Drawing for the job (mm, zero at the part's lowest x, y, z). A direction names the side the tool comes from. Coordinates: 2 decimals unless noted, no trailing zeros. Order: outer loops, then holes, each group sorted by start corner. A loop starts at its lowest first (then second) coordinate and runs counter-clockwise, first axis right, second up. Notation, with made-up numbers: (15, 62.5) - (72, 62.5) arc R17 cw to (72, 78.5) - close; hole circle Ø2 at (-35.75, -28). An arc over 180 degrees is marked (long way). Answer as CSV lines item,"result". Start each with the question number.
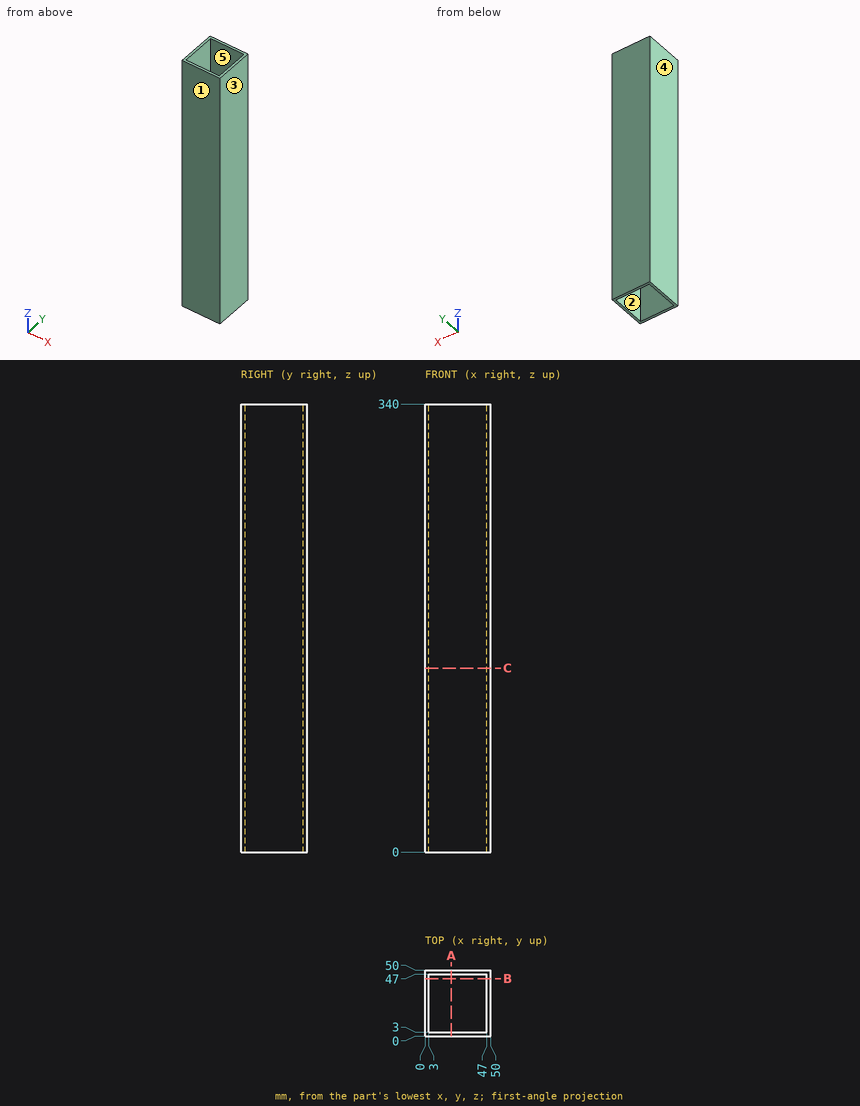
(1) Which spindle directions (+Z, -Z, +X, -X, +Y, -Y) get a long thin tool onto all of the face, cutting with end or side? Do the marked faces 4 and 5. Say none if no direction does.
(2) Band-saw the part on A-A on x = 20. List the corners of the cut face in (y, z), plus the area to 3 significant figures.
(3) Probe L1, parallel to Y at x = 19.5, z = 121.5. List the from-to ranges inside material, lowest first. Write a range as [from, to].
(4) Pull direction Y, two halves, no side cores. Call the marked faces 1, 2 and 3: +Y half, -Y half, draft (parallel to the pull), parting line (faces both ways), or undercut.
(5) Band-saw the part on C-C on z = 139.5. List the corners of the cut face in (x, y).
Filled in:
1,face 4,"+Z, -Z, -X, +Y, -Y"
1,face 5,"+Z, -Z"
2,outline,"(0, 0) - (3, 0) - (3, 340) - (0, 340) - close; (47, 0) - (50, 0) - (50, 340) - (47, 340) - close"
2,area,"2,040 mm^2"
3,L1,"y = [0, 3], [47, 50]"
4,face 1,"-Y half"
4,face 2,"undercut"
4,face 3,"draft"
5,outline,"(0, 0) - (50, 0) - (50, 50) - (0, 50) - close; hole (3, 3) - (47, 3) - (47, 47) - (3, 47) - close"
